Build history of the part. All positions in model axes, mm. A direction names the side the tool comes from. Give positions to 0.01 mm unless a question says otherwise; leave off trailing zeros. Order: outer loops, then holes, each group sorted by start corner. A loop starts at its lowest first (then second) coordinate and runs counter-clockwise, first axis right, second up. Notation, with made-up numbers: (81.5, -27) - (107.5, -27) arc R20 cw to (107.5, -19) - close; hole circle Ø6 at (21.5, 33.25). An arc over 180 degrees is marked (long way). Answer in a Markdown table with one row per item.
```python
from build123d import *

# Parameters (mm, degrees)
CHAMFER1_SIZE         = 0.24
CUT_EXTRUDE1_DEPTH    = 3
BODY_MOVE_COPY1_ANGLE = 180


with BuildPart() as part:
    # Sketch2 → Revolve1 (revolve)
    with BuildSketch(Plane.XY):
        Polygon((2, -4), (2, -1), (0, 0.154700538), (0, 8), (3, 8), (3, 0), (5, 0), (5, -4), align=None)
    revolve(axis=Axis((0, 0.154700538, 0), (0, 1, 0)))

    # Chamfer1
    chamfer1_edges = [part.edges().sort_by_distance(p)[0] for p in [
        (-5, -4, 0),
        (-3, 8, 0),
    ]]
    chamfer(chamfer1_edges, length=CHAMFER1_SIZE)

    # Sketch3 → Cut-Extrude1 (cut)
    with BuildSketch(Plane.XZ.offset(4)):
        Polygon((-1.154700538, 2), (-2.309401077, 0), (-1.154700538, -2), (1.154700538, -2), (2.309401077, 0), (1.154700538, 2), align=None)
    extrude(amount=-CUT_EXTRUDE1_DEPTH, mode=Mode.SUBTRACT)


with BuildPart() as part_1:
    # Body-Move/Copy1: moved
    add(part.part.rotate(Axis((0, 3.25, 0), (1, 0, 0)), BODY_MOVE_COPY1_ANGLE))


solid = part_1.part
```
1. Which spindle directions (+Z, -Z, +X, -X, +Y, -Y) get a long thin tool onto all of the face, cutting with end or side? Do faces 1 (the face through (1.724, 9.021, 1.014)), 2 (the face through (2, 10.5, -1)), 3 (the face through (-3.3, 6.5, 0.1)). Say none if no direction does.
Check result:
| item | result |
|---|---|
| face 1 | +Y |
| face 2 | +Z, -Z, +X, -X, +Y |
| face 3 | -Y |
2. Drop flat-ended pins along their axis: P1, Ø1.1, axis at x = -0.5, z = -1.5, coming from the +Y side; P2, Ø0.5, axis at x = 0.5, z = 1.5, coming from the +Y side; P3, Ø5, axis at y = 1, z = 3.5, coming from the +X side; P4, Ø1, axis at x = -3, y = 4.5, coming from the +Z side. Give the stop position or say it passes through.
Check result:
| item | result |
|---|---|
| P1 | stops at y = 10.5 |
| P2 | stops at y = 7.4 |
| P3 | stops at x = 2.83 |
| P4 | stops at z = 1.66 |
3. Probe line 1 (Y direction, x = -2.5, z = -3); line 2 (Z direction, x = 0, y = 5); line 3 (Y direction, x = -1, z = -1.75). List the from-to ranges inside material, lowest first.
Check result:
| item | result |
|---|---|
| line 1 | y = 6.5 to 10.5 |
| line 2 | z = -3 to 3 |
| line 3 | y = -1.5 to 7.5 |
4. Cut at A-A on y = 9. Write the cut outline in (x, z).
Check result:
| item | result |
|---|---|
| outline | circle Ø10 at (0, 0); hole (-2.31, 0) - (-1.15, -2) - (1.15, -2) - (2.31, 0) - (1.15, 2) - (-1.15, 2) - close |
5. Two-plate mould, pull along Z, no slides. Class faces 4 (the face through (-3, 3, 0)), 5 (the face through (0, -1.5, 0)), 6 (the face through (-1.724, 9.021, -1.014)), 7 (the face through (1.74, 9.02, -0.99)): +Z half, -Z half, draft (parallel to the pull), parting line (faces both ways), or undercut.
Check result:
| item | result |
|---|---|
| face 4 | parting line |
| face 5 | draft |
| face 6 | undercut |
| face 7 | undercut |
6. Cut at B-B on y = 2.5. Write the cut outline in (x, z).
Check result:
| item | result |
|---|---|
| outline | circle Ø6 at (0, 0) |
